from build123d import *

# Parameters (mm, degrees)
EDGE_CHAMFER_0_025IN_X_45DEG_SIZE  = 0.635
DRILLED_HOLE_0_5_X_0_75_DEEP_D     = 12.7
DRILLED_HOLE_0_5_X_0_75_DEEP_DEPTH = 19.05
DRILLED_HOLE_0_5_X_0_75_DEEP_TIP   = 3.815464931


with BuildPart() as part:
    # Turned Profile Sketch → Turned Body (revolve)
    with BuildSketch(Plane.XY):
        Polygon((0, 0), (0, 25.4), (-25.4, 25.4), (-25.4, 19.05), (-44.45, 19.05), (-44.45, 0), (-0.941021968, 0), align=None)
    revolve(axis=Axis((-0.941021968, 0, 0), (-1, 0, 0)))

    # Sketch4 → Tapped Hole 1-4-20 x 0.5 Deep (revolve, cut)
    with BuildSketch(Plane(origin=(-44.45, 0, 0), x_dir=(0, 0, 1), z_dir=(0, 1, 0))):
        Polygon((0, 0), (0, 20.583816902), (2.5527, 19.05), (2.5527, 12.7), (3.175, 12.7), (3.175, 0.730483939), (3.81, 0), align=None)
    revolve(axis=Axis((-50.8, 0, 0), (1, 0, 0)), mode=Mode.SUBTRACT)

    # Edge Chamfer 0.025in x 45deg
    edge_chamfer_0_025in_x_45deg_edges = [part.edges().sort_by_distance(p)[0] for p in [
        (-44.45, -19.05, 0),
    ]]
    chamfer(edge_chamfer_0_025in_x_45deg_edges, length=EDGE_CHAMFER_0_025IN_X_45DEG_SIZE)

    # Drilled Hole Ø0.5 x 0.75 Deep
    with Locations(Plane.YZ):
        with Locations((0, 0)):
            Hole(DRILLED_HOLE_0_5_X_0_75_DEEP_D / 2, depth=DRILLED_HOLE_0_5_X_0_75_DEEP_DEPTH)
            with Locations((0, 0, -(DRILLED_HOLE_0_5_X_0_75_DEEP_DEPTH + DRILLED_HOLE_0_5_X_0_75_DEEP_TIP / 2))):  # 118° drill point
                Cone(0, DRILLED_HOLE_0_5_X_0_75_DEEP_D / 2, DRILLED_HOLE_0_5_X_0_75_DEEP_TIP, mode=Mode.SUBTRACT)


solid = part.part
Part model, mm, in its own coordinate system. A direction names the side the tool comes from. Give positions to 0.01 mm unless a question says otherwise; leave off trailing zeros. Loops run counter-clockwise (first coordinate to the right, second up) from the corner with the lowest first, then second, coordinate; pieces in that order, holes last.
(1) Pin check, flat tips, straight feed: pin 1 (10 mm diameter, centred on y = 0, z = 0, fed in from -X); pin 2 (4 mm diameter, centred on x = -18.5, y = 9.5, fed in from +Z); pin 3 (10 mm diameter, centred on x = -16.5, y = -4, fed in from +Z); pin 4 (1 mm diameter, centred on x = -8, z = -3.5, fed in from +Y). Stop position of each tip, or through.
Return value:
pin 1: stops at x = -44.45
pin 2: stops at z = 24.27
pin 3: stops at z = 25.4
pin 4: stops at y = 25.22
(2) 3-axis set-ups, long thin cutter, end or side, ignore diameter. For faces 1 (the cylindrical face through (-9.66, 1.38, -6.2)), 2 (the flat face through (0, -5, 5)), 3 (the cylindrical face through (-37.82, 3.1, -0.69)): which of +Z, -Z, +X, -X, +Y, -Y reach the whole face in a straight line?
Return value:
face 1: +X
face 2: +Z, -Z, +X, +Y, -Y
face 3: -X
(3) Band-saw the part on A-A (x = -29.5). Write the cut outline in (y, z).
Return value:
outline: circle Ø38.1 at (0, 0); hole circle Ø5.11 at (0, 0)
(4) Pull direction Y, two halves, no side cores. Call faces 4 (the flat face through (-44.45, 0, 4)), 5 (the cylindrical face through (-28.619, -0.767, 2.435)), 6 (the cylindrical face through (-12.878, -5.506, 24.796)): pulls with the +Y half, pulls with the -Y half, needs draft (parallel to the pull), parting line crosses it, or undercut.
Return value:
face 4: needs draft
face 5: undercut
face 6: parting line crosses it
(5) Band-saw the part on B-B (x = -14). Write the cut outline in (y, z), and give its area (3 significant figures).
Return value:
outline: circle Ø50.8 at (0, 0); hole circle Ø12.7 at (0, 0)
area: 1,900 mm2
(6) Drill centre lines: line 1 along Y through (x, z) = (-4, 0); line 2 along Y through (x, z) = (-30, 0). Where is each one in solid material? Low to high.
Return value:
line 1: y = -25.4 to -6.35, 6.35 to 25.4
line 2: y = -19.05 to -2.55, 2.55 to 19.05
